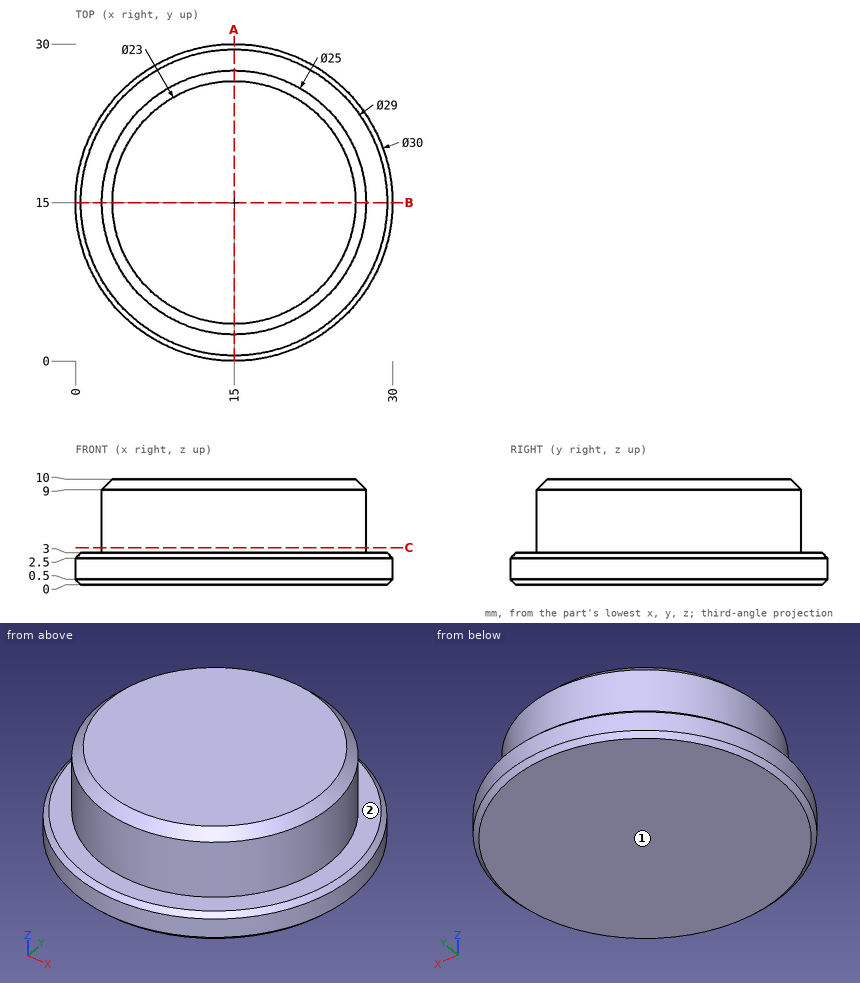
Check sheet for the drawn part. Datum: minimum x, y, z corner. Units: mm. A direction names the side the tool comes from. Give positions to 0.01 mm unless a question says otherwise; leave off trailing zeros. Order: outer loops, then holes, each group sorted by start corner. A loop starts at its lowest first (then second) coordinate and runs counter-clockwise, first axis right, second up. Notation, with made-up numbers: (60.5, -21.75) -> (72.5, -21.75) arc R14 cw to (72.5, 1.25) -> close; hole circle Ø2 at (16.25, -15.5). An arc over 180 degrees is marked (long way). Use a Markdown table: item, result.
1) Section check A-A, the plane x = 15. Record the boundary of the cut face in (y, z), then the cut area to 4 significant figures.
Results:
| item | result |
|---|---|
| outline | (0, 0.5) -> (0.5, 0) -> (29.5, 0) -> (30, 0.5) -> (30, 2.5) -> (29.5, 3) -> (27.5, 3) -> (27.5, 9) -> (26.5, 10) -> (3.5, 10) -> (2.5, 9) -> (2.5, 3) -> (0.5, 3) -> (0, 2.5) -> close |
| area | 263.5 mm² |
2) Tool access check on the marked faces 1 and 2. Record the directions out of +Z, -Z, +X, -X, +Y, -Y that give a thin tool (end or side, any length) a straight path to the whole face; none if there is none.
Results:
| item | result |
|---|---|
| face 1 | -Z, +X, -X, +Y, -Y |
| face 2 | +Z |
3) Material ranges on probe 1 along Z at (x, y) = (25, 6.5); probe 2 along X at (y, z) = (25, 9.25); probe 3 along X at (y, z) = (26, 4), recorded low to high.
Results:
| item | result |
|---|---|
| probe 1 | 0 to 3 |
| probe 2 | 7.92 to 22.08 |
| probe 3 | 9.06 to 20.94 |
4) Depth check by flat-ended pin: pin 1 Ø5 at (x, z) = (10.5, 7) entering from -Y; pin 2 Ø1.5 at (x, y) = (24, 23.5) entering from +Z; pin 3 Ø2 at (x, y) = (12, 21) entering from -Z; pin 4 Ø6 at (y, z) = (17, 6.5) entering from -X. Enter the tip coordinate at first touch or a pass-through.
Results:
| item | result |
|---|---|
| pin 1 | y = 2.66 |
| pin 2 | z = 9.87 |
| pin 3 | z = 0 |
| pin 4 | x = 2.5 |
5) Section check C-C, the plane z = 3.5. Record the boundary of the cut face in (x, y).
Results:
| item | result |
|---|---|
| outline | circle Ø25 at (15, 15) |
